```python
from build123d import *

# Parameters (mm, degrees)
EXTRUDE_1_DEPTH     = 60
SKETCH_2_R          = 10
CUT_EXTRUDE_1_DEPTH = 78.808619714
SKETCH_3_R          = 2.1
CUT_EXTRUDE_2_DEPTH = 78.808619714
SKETCH_4_R          = 2.75
CUT_EXTRUDE_3_DEPTH = 81.17516917
SKETCH_5_R          = 5
CUT_EXTRUDE_4_DEPTH = 5.8


with BuildPart() as part:
    # 草图1 → 凸台-拉伸1 (new body)
    with BuildSketch(Plane.XY):
        Polygon((-12.892307692, 45.323076923), (-12.892307692, -2.676923077), (7.107692308, -2.676923077), (7.107692308, -14.676923077), (-22.892307692, -14.676923077), (-22.892307692, 45.323076923), align=None)
    extrude(amount=EXTRUDE_1_DEPTH)

    # 草图2 → 切除-拉伸1 (cut, through all)
    with BuildSketch(Plane(origin=(-12.892307692, 0, 0), x_dir=(0, 0, -1), z_dir=(1, 0, 0))):
        with Locations(Location((-30, 15.323076923, 0), (0, 0, 90))):
            Circle(SKETCH_2_R)
    extrude(amount=-CUT_EXTRUDE_1_DEPTH, mode=Mode.SUBTRACT)

    # 草图3 → 切除-拉伸2 (cut, through all)
    with BuildSketch(Plane(origin=(-12.892307692, 0, 0), x_dir=(0, 0, -1), z_dir=(1, 0, 0))):
        with Locations(Location((-54.75, 40.073076923, 0), (0, 0, 90))):
            Circle(SKETCH_3_R)
        with Locations(Location((-5.25, 40.073076923, 0), (0, 0, 90))):
            Circle(SKETCH_3_R)
    extrude(amount=-CUT_EXTRUDE_2_DEPTH, mode=Mode.SUBTRACT)

    # 草图4 → 切除-拉伸3 (cut, through all)
    with BuildSketch(Plane(origin=(0, -2.676923077, 0), x_dir=(1, 0, 0), z_dir=(0, 1, 0))):
        with Locations(Location((-2.892307692, -10, 0), (0, 0, 270))):
            Circle(SKETCH_4_R)
        with Locations(Location((-2.892307692, -50, 0), (0, 0, 270))):
            Circle(SKETCH_4_R)
    extrude(amount=-CUT_EXTRUDE_3_DEPTH, mode=Mode.SUBTRACT)

    # 草图5 → 切除-拉伸4 (cut)
    with BuildSketch(Plane(origin=(0, -2.676923077, 0), x_dir=(1, 0, 0), z_dir=(0, 1, 0))):
        with Locations(Location((-2.892307692, -10, 0), (0, 0, 270))):
            Circle(SKETCH_5_R)
        with Locations(Location((-2.892307692, -50, 0), (0, 0, 270))):
            Circle(SKETCH_5_R)
    extrude(amount=-CUT_EXTRUDE_4_DEPTH, mode=Mode.SUBTRACT)


solid = part.part
```
Here's how the part is built. I have some questions about the finished solid (model axes, mm). A direction names the side the tool comes from. Round coordinates to 2 decimals unless told otherwise and drop trailing zeros. Loops run counter-clockwise (first coordinate to the right, second up) from the corner with the lowest first, then second, coordinate; pieces in that order, holes last. Notation, with made-up numbers: (36.25, -1) -> (61.25, -1) arc R16 cw to (61.25, 13) -> close; hole circle Ø8 at (35.25, -8.5). An arc over 180 degrees is marked (long way). Answer as CSV lines item,"result".
1. If we section it at D-D on z = 30: Please give me the cut outline in (x, y).
Final values:
outline,"(-22.89, -14.68) -> (7.11, -14.68) -> (7.11, -2.68) -> (-12.89, -2.68) -> (-12.89, 5.32) -> (-22.89, 5.32) -> close; (-22.89, 25.32) -> (-12.89, 25.32) -> (-12.89, 45.32) -> (-22.89, 45.32) -> close"
2. If I drill on L1, parallel to X at y = -6, z = 10; L2, parallel to X at y = 8.5, z = 13.5; L3, parallel to Y at x = 1, z = 38, over which ranges is the centre line in solid material (lowest first)?
Final values:
L1,"x = -22.89 to -7.89, 2.11 to 7.11"
L2,"x = -22.89 to -12.89"
L3,"y = -14.68 to -2.68"
3. Thinking about a two-plate mould opening in X: for faces 4 (the face through (-5, -8.477, 12)), 5 (the face through (-14, 9, 60)), 6 (the face through (-12.892, 27, 30)), which applies, released by +X, released by -X, zero draft, split by the parting line, or undercut?
Final values:
face 4,"undercut"
face 5,"zero draft"
face 6,"released by +X"
4. If we section it at B-B on x = -18.25: Please give me the cut outline in (y, z), plus the area to 3 significant figures.
Final values:
outline,"(-14.68, 0) -> (45.32, 0) -> (45.32, 60) -> (-14.68, 60) -> close; hole circle Ø20 at (15.32, 30); hole circle Ø4.2 at (40.07, 5.25); hole circle Ø4.2 at (40.07, 54.75)"
area,"3,260 mm^2"
5. If we section it at C-C on y = 18: Please give me the cut outline in (x, z), plus the area to 3 significant figures.
Final values:
outline,"(-22.89, 0) -> (-12.89, 0) -> (-12.89, 20.36) -> (-22.89, 20.36) -> close; (-22.89, 39.64) -> (-12.89, 39.64) -> (-12.89, 60) -> (-22.89, 60) -> close"
area,"407 mm^2"
6. Which directions (+Z, -Z, +X, -X, +Y, -Y) give clear straight access to the entire face, cutting with the end or side of a thin tool? Please do faces 1 (the face through (-17.822, 13.155, 20.238)), 2 (the face through (-3, -2.677, 30)), 3 (the face through (-1.39, -5.54, 14.77)).
Final values:
face 1,"+X, -X"
face 2,"+Z, -Z, +X, +Y"
face 3,"+Y"
7. For pin 1 (10 mm diameter, centred on x = -10, z = 32, fed in from +Y); pin 2 (6.5 mm diameter, centred on x = -2.89, z = 50, fed in from +Y); pin 3 (11 mm diameter, centred on x = -3, z = 48.5, fed in from +Y); pin 4 (24 mm diameter, centred on y = 12, z = 26.5, fed in from +X), each with a flat end and sliding along its axis, tell me the tip position at first contact or that it passes through.
Final values:
pin 1,"stops at y = 45.32"
pin 2,"stops at y = -8.48"
pin 3,"stops at y = -2.68"
pin 4,"stops at x = -12.89"
8. If we section it at A-A on z = 10: Please give me the cut outline in (x, y).
Final values:
outline,"(-22.89, -14.68) -> (-5.64, -14.68) -> (-5.64, -8.48) -> (-7.89, -8.48) -> (-7.89, -2.68) -> (-12.89, -2.68) -> (-12.89, 45.32) -> (-22.89, 45.32) -> close; (-0.14, -14.68) -> (7.11, -14.68) -> (7.11, -2.68) -> (2.11, -2.68) -> (2.11, -8.48) -> (-0.14, -8.48) -> close"
